Here's how the part is built. I have some questions about the finished solid (model axes, mm). Coordinates: 2 decimals unless noted, no trailing zeros. Write each loop counter-clockwise with the first axis right and the second up, starting at its lowest first coordinate (ties: lowest second). Pieces come first, ordered by that corner, then holes. Notation, with made-up numbers: (67.25, 11.5) - (112.25, 11.5) arc R33 cw to (112.25, 44.5) - close; hole circle Ø10 at (31, 41.5). An arc over 180 degrees is marked (long way). Answer in a Markdown table with one row per item. Add a question column.
Item 1: Imagine slicing it at A-A (z = 2.5). Please give me the cut outline in (x, y), plus the area to 4 significant figures.
Item 2: I'm going to push a flat-ended pin straight in: pin 1 (2 mm diameter, centred on y = 99, z = -4.5, fed in from +X). Where does the tip first touch, or does it pass through?
Item 3: Imagine slicing it at B-B (y = 97). Please give me the cut outline in (x, z), plus the area to 3 significant figures.
Item 4: Imagine slicing it at C-C (x = 112.5). Please give me the cut outline in (y, z), plus the area to 3 significant figures.
Item 5: We'd pull the mould along Z, two halves only. Please class faces 1 (the face through (59, 66, -8)), 2 (the face through (59, 66, 8)), 3 (the face through (95, 105, 0)): +Z half, -Z half, draft (parallel to the pull), parting line (faces both ways), or undercut.
Item 6: If I drill on probe 1 along X at (y, z) = (104.5, -6.75); probe 2 along Y at (x, z) = (90, -6); probe 3 along X at (y, z) = (84, 3), over which ranges is the centre line in solid material (lowest first)? Write a range as from..to.
from build123d import *

# Parameters (mm, degrees)
SKETCH1_W           = 120
SKETCH1_H           = 130
BOSS_EXTRUDE1_DEPTH = 8
CHAMFER1_SIZE       = 50


with BuildPart() as part:
    # Sketch1 → Boss-Extrude1 (new, symmetric)
    with BuildSketch(Plane.XY):
        with Locations((60, 65)):
            Rectangle(SKETCH1_W, SKETCH1_H)
    extrude(amount=BOSS_EXTRUDE1_DEPTH, both=True)

    # Chamfer1
    chamfer1_edges = [part.edges().sort_by_distance(p)[0] for p in [
        (120, 130, 0),
    ]]
    chamfer(chamfer1_edges, length=CHAMFER1_SIZE)


solid = part.part
Here are the results:
| question | item | result |
|---|---|---|
| 1 | outline | (0, 0) - (120, 0) - (120, 80) - (70, 130) - (0, 130) - close |
| 1 | area | 14,350 mm2 |
| 2 | pin 1 | stops at x = 102 |
| 3 | outline | (0, -8) - (103, -8) - (103, 8) - (0, 8) - close |
| 3 | area | 1,650 mm2 |
| 4 | outline | (0, -8) - (87.5, -8) - (87.5, 8) - (0, 8) - close |
| 4 | area | 1,400 mm2 |
| 5 | face 1 | -Z half |
| 5 | face 2 | +Z half |
| 5 | face 3 | draft |
| 6 | probe 1 | x = 0..95.5 |
| 6 | probe 2 | y = 0..110 |
| 6 | probe 3 | x = 0..116 |
